Design review of the part built by this model. Coordinates are the model's own, in mm. Face numbers are marked on the shaded views. Give positions to 0.01 mm unless a question says otherwise; leave off trailing zeros. Loops run counter-clockwise (first coordinate to the right, second up) from the corner with the lowest first, then second, coordinate; pieces in that order, holes last. Notation, with made-up numbers: (47.25, 14) -> (85.25, 14) arc R19 cw to (85.25, 45) -> close; hole circle Ø8 at (-12, 8). An arc over 180 degrees is marked (long way). Use a Markdown table: item, result. Add a question column.
1. Draft analysis for pull direction Z (two halves, no side actions). For the marked faces 1, 2 and 3, state which applies: pulls with the +Z half, pulls with the -Z half, needs draft (parallel to the pull), parting line crosses it, or undercut.
2. Add section B-B (y = 0). State the section outline as (x, z) points, and give its area (3 significant figures).
3. To check wall thickness, follow line 1 (Y direction, x = 0, z = 11); line 2 (X direction, y = -22, z = 6.75); line 3 (X direction, y = -21, z = 6.75). State the ranges of each line that lie inside material, in increasing order.
4. For pin 1 Ø3 at (y, z) = (-8.5, 7.5) entering from -X; pin 2 Ø5 at (y, z) = (29, 5.5) entering from +X; pin 3 Ø3 at (x, z) = (30, 12.5) entering from +Y; pin 4 Ø7 at (x, y) = (34.64, -20) entering from +Z, all flat-tipped, find the tip position at first contact; note any pin that passes through.
5. Add section A-A (x = 0). State the section outline as (y, z) points.
6. Add section C-C (z = 7). State the section outline as (x, y) points (3 decimals), and give its area (3 significant figures).
```python
from build123d import *

# Parameters (mm, degrees)
SKETCH1_R           = 50
SKETCH1_R_2         = 20
BOSS_EXTRUDE1_DEPTH = 16
CIRPATTERN1_COUNT   = 3
CHAMFER1_SIZE       = 0.2


with BuildPart() as part:
    # Sketch1 → Boss-Extrude1 (new body)
    with BuildSketch(Plane.XY):
        Circle(SKETCH1_R)
        Circle(SKETCH1_R_2, mode=Mode.SUBTRACT)
    extrude(amount=BOSS_EXTRUDE1_DEPTH)

    # Sketch5 → M10 Tapped Hole1 (revolve, cut)
    with BuildSketch(Plane(origin=(0, 40, 16), x_dir=(0, -1, 0), z_dir=(1, 0, 0))):
        Polygon((0, 0), (0, 31.803657631), (4.25, 29.25), (4.25, 0), align=None)
    m10_tapped_hole1 = revolve(axis=Axis((0, 40, 22.35), (0, 0, -1)), mode=Mode.SUBTRACT)

    # CirPattern1: M10 Tapped Hole1 ×3 about axis
    cirpattern1_axis = Axis((0, 0, 0), (0, 0, 1))
    for i in range(1, CIRPATTERN1_COUNT):
        add(m10_tapped_hole1.rotate(cirpattern1_axis, i * 360 / CIRPATTERN1_COUNT), mode=Mode.SUBTRACT)

    # Chamfer1
    chamfer1_edges = [part.edges().sort_by_distance(p)[0] for p in [
        (-50, 0, 0),
        (-50, 0, 16),
        (-20, 0, 0),
        (-20, 0, 16),
    ]]
    chamfer(chamfer1_edges, length=CHAMFER1_SIZE)


solid = part.part
```
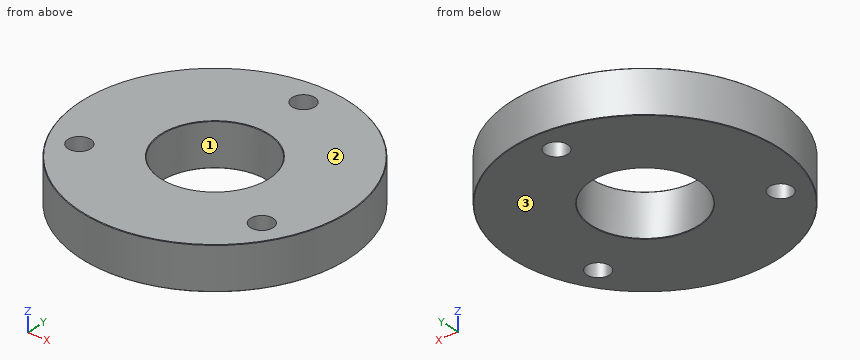
Taken from the geometry:
| question | item | result |
|---|---|---|
| 1 | face 1 | needs draft |
| 1 | face 2 | pulls with the +Z half |
| 1 | face 3 | pulls with the -Z half |
| 2 | outline | (-50, 0.2) -> (-49.8, 0) -> (-20.2, 0) -> (-20, 0.2) -> (-20, 15.8) -> (-20.2, 16) -> (-49.8, 16) -> (-50, 15.8) -> close; (20, 0.2) -> (20.2, 0) -> (49.8, 0) -> (50, 0.2) -> (50, 15.8) -> (49.8, 16) -> (20.2, 16) -> (20, 15.8) -> close |
| 2 | area | 960 mm^2 |
| 3 | line 1 | y = -50 to -20, 20 to 35.75, 44.25 to 50 |
| 3 | line 2 | x = -44.9 to -38.39, -30.89 to 30.89, 38.39 to 44.9 |
| 3 | line 3 | x = -45.38 to -38.77, -30.51 to 30.51, 38.77 to 45.38 |
| 4 | pin 1 | stops at x = -49.51 |
| 4 | pin 2 | stops at x = 42.4 |
| 4 | pin 3 | stops at y = 41.08 |
| 4 | pin 4 | passes through |
| 5 | outline | (-50, 0.2) -> (-49.8, 0) -> (-20.2, 0) -> (-20, 0.2) -> (-20, 15.8) -> (-20.2, 16) -> (-49.8, 16) -> (-50, 15.8) -> close; (20, 0.2) -> (20.2, 0) -> (35.75, 0) -> (35.75, 16) -> (20.2, 16) -> (20, 15.8) -> close; (44.25, 0) -> (49.8, 0) -> (50, 0.2) -> (50, 15.8) -> (49.8, 16) -> (44.25, 16) -> close |
| 6 | outline | circle Ø100 at (0, 0); hole circle Ø8.5 at (-34.641, -20); hole circle Ø40 at (0, 0); hole circle Ø8.5 at (0, 40); hole circle Ø8.5 at (34.641, -20) |
| 6 | area | 6,430 mm^2 |
